For this review, take the finished solid that the model builds, in its own axes (mm). Face numbers are marked on the shaded views. A direction names the side the tool comes from. Round coordinates to 2 decimals unless told otherwise and drop trailing zeros. Order: outer loops, then holes, each group sorted by start corner. A loop starts at its lowest first (then second) coordinate and runs counter-clockwise, first axis right, second up. Notation, with made-up numbers: M -27.75,83 L 22.25,83 A32 ccw 22.25,120 Z; hole C -22.5,75 d10. An arc over 180 degrees is marked long. Answer as a JSON object with one key per item and string values.
from build123d import *

# Parameters (mm, degrees)
SKETCH_1_R             = 25
EXTRUDE_1_DEPTH        = 30
SKETCH_2_R             = 30
EXTRUDE_2_DEPTH        = 30
SKETCH_4_R             = 15
CUT_EXTRUDE_1_DEPTH    = 74.484692283
EXTRUDE_START          = -30
SKETCH_13_R            = 15
EXTRUDE_4_DEPTH        = 30
SKETCH_12_R            = 17.5
EXTRUDE_3_DEPTH        = 32
HOLE_WIZARD_M6_1_D     = 5
HOLE_WIZARD_M6_1_DEPTH = 15
HOLE_WIZARD_M6_1_TIP   = 1.502151548
CUT_EXTRUDE_START      = -13
SKETCH_16_R            = 17.5
SKETCH_16_R_2          = 15
CUT_EXTRUDE_3_DEPTH    = 13
CHAMFER_4_SIZE         = 1


with BuildPart() as part:
    # 草图1 → 凸台-拉伸1 (new body)
    with BuildSketch(Plane.XY):
        Circle(SKETCH_1_R)
    extrude(amount=EXTRUDE_1_DEPTH)

    # 草图2 → 凸台-拉伸2 (add)
    with BuildSketch(Plane.XY.offset(30)):
        Circle(SKETCH_2_R)
    extrude(amount=EXTRUDE_2_DEPTH)

    # 草图4 → 切除-拉伸1 (cut, through all)
    with BuildSketch(Plane(origin=(0, 0, 0), x_dir=(-1, 0, 0), z_dir=(0, 0, -1))):
        Circle(SKETCH_4_R)
    extrude(amount=-CUT_EXTRUDE_1_DEPTH, mode=Mode.SUBTRACT)

    # 草图13 → 凸台-拉伸4 (add)
    with BuildSketch(Plane.XY.offset(60).offset(EXTRUDE_START)):
        with Locations(Location((0, 0, 0), (0, 0, 180))):
            Circle(SKETCH_13_R)
    extrude(amount=EXTRUDE_4_DEPTH)

    # 草图12 → 凸台-拉伸3 (add)
    with BuildSketch(Plane.XY.offset(60)):
        Circle(SKETCH_12_R)
    extrude(amount=EXTRUDE_3_DEPTH)

    # M6 螺纹孔1
    with Locations(Plane.XY.offset(92)):
        with Locations((0, 0)):
            Hole(HOLE_WIZARD_M6_1_D / 2, depth=HOLE_WIZARD_M6_1_DEPTH)
            with Locations((0, 0, -(HOLE_WIZARD_M6_1_DEPTH + HOLE_WIZARD_M6_1_TIP / 2))):  # 118° drill point
                Cone(0, HOLE_WIZARD_M6_1_D / 2, HOLE_WIZARD_M6_1_TIP, mode=Mode.SUBTRACT)

    # 草图16 → 切除-拉伸3 (cut)
    with BuildSketch(Plane.XY.offset(92).offset(CUT_EXTRUDE_START)):
        Circle(SKETCH_16_R)
        with Locations(Location((0, 0, 0), (0, 0, 180))):
            Circle(SKETCH_16_R_2, mode=Mode.SUBTRACT)
    extrude(amount=CUT_EXTRUDE_3_DEPTH, mode=Mode.SUBTRACT)

    # 倒角4
    chamfer_4_edges = [part.edges().sort_by_distance(p)[0] for p in [
        (15, 0, 0),
        (15, 0, 92),
        (-30, 0, 30),
        (-30, 0, 60),
    ]]
    chamfer(chamfer_4_edges, length=CHAMFER_4_SIZE)


solid = part.part
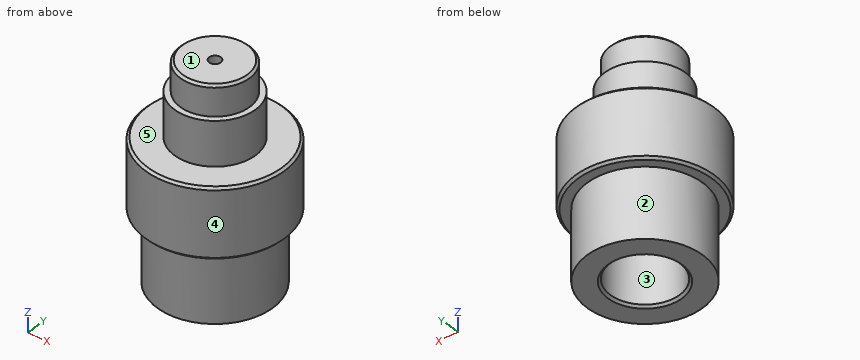
1) Add section B-B on z = 64. State the section outline as (x, y) points.
Geometry check:
{"outline": "C 0,0 d35"}
2) Mouldability with a two-part tool opening along X and no side actions: class the marked faces 1, 2 and 3 as +X half, -X half, draft (parallel to the pull), parting line (faces both ways), or undercut.
Geometry check:
{"face 1": "draft", "face 2": "parting line", "face 3": "undercut"}
3) Add section A-A on z = 23. State the section outline as (x, y) points.
Geometry check:
{"outline": "C 0,0 d50; hole C 0,0 d30"}
4) For L1, parallel to Y at x = 0, z = 9; L2, parallel to Y at x = 0, z = 84; L3, parallel to Z at x = -13.5, y = -10, list the stretches that pass through material, from the lowest coordinate up.
Geometry check:
{"L1": "y = -25 to -15, 15 to 25", "L2": "y = -15 to -2.5, 2.5 to 15", "L3": "z = 0 to 79"}
5) Add section C-C on z = 83.5. State the section outline as (x, y) points, and give its area (3 significant figures).
Geometry check:
{"outline": "C 0,0 d30; hole C 0,0 d5", "area": "687 mm²"}
6) Machinability: for the marked faces 4 and 5, which of the approach directions +Z, -Z, +X, -X, +Y, -Y give a long, thin tool a straight path to every point of the face, cutting with its end or side? Answer none if there is none.
Geometry check:
{"face 4": "+Z, -Z", "face 5": "+Z"}
7) Insertion check: P1, Ø10, axis at x = -16.5, y = -11, coming from the +Z side; P2, Ø4, axis at y = -13.5, z = 11, coming from the +X side; P3, Ø6, axis at x = -21.5, z = 20.5, coming from the -Y side. Each pin has a flat end and moves straight along its axis. Give the tip position at first contact, or say it passes through.
Geometry check:
{"P1": "stops at z = 91.17", "P2": "stops at x = 22.2", "P3": "stops at y = -16.82"}
